from build123d import *

# Parameters (mm, degrees)
M10X1_0_TAPPED_HOLE1_D     = 9
M10X1_0_TAPPED_HOLE1_DEPTH = 28
M10X1_0_TAPPED_HOLE1_TIP   = 2.703872786
M4_TAPPED_HOLE1_D          = 3.3
M4_TAPPED_HOLE1_DEPTH      = 10.1
M4_TAPPED_HOLE1_TIP        = 0.991420021


with BuildPart() as part:
    # Sketch1 → Revolve1 (revolve)
    with BuildSketch(Plane.XY, mode=Mode.PRIVATE) as revolve1_sk:
        Polygon((0, 0), (-9, 0), (-9, 18), (-15, 36), (-15, 50), (-13.5, 50), (-13.5, 45), (0, 45), align=None)
    revolve(revolve1_sk.sketch.rotate(Axis((0, 0, 0), (0, -1, 0)), 270), axis=Axis((0, 0, 0), (0, -1, 0)))

    # M10x1.0 Tapped Hole1
    with Locations(Plane(origin=(0, 0, 0), x_dir=(-1, 0, 0), z_dir=(0, -1, 0))):
        with Locations((0, 0)):
            Hole(M10X1_0_TAPPED_HOLE1_D / 2, depth=M10X1_0_TAPPED_HOLE1_DEPTH)
            with Locations((0, 0, -(M10X1_0_TAPPED_HOLE1_DEPTH + M10X1_0_TAPPED_HOLE1_TIP / 2))):  # 118° drill point
                Cone(0, M10X1_0_TAPPED_HOLE1_D / 2, M10X1_0_TAPPED_HOLE1_TIP, mode=Mode.SUBTRACT)

    # M4 Tapped Hole1
    with Locations(Plane(origin=(0, 45, 0), x_dir=(1, 0, 0), z_dir=(0, 1, 0))):
        with Locations((0, 0)):
            Hole(M4_TAPPED_HOLE1_D / 2, depth=M4_TAPPED_HOLE1_DEPTH)
            with Locations((0, 0, -(M4_TAPPED_HOLE1_DEPTH + M4_TAPPED_HOLE1_TIP / 2))):  # 118° drill point
                Cone(0, M4_TAPPED_HOLE1_D / 2, M4_TAPPED_HOLE1_TIP, mode=Mode.SUBTRACT)


solid = part.part
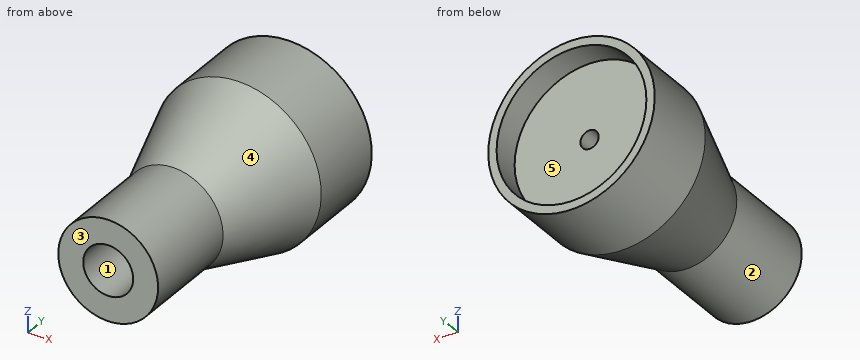
Source: CAD feature listing. Evaluate the final solid. Frame: model axes, mm. Face numbers are marked on the shaded views. A direction names the side the tool comes from. Coordinates: 2 decimals unless noted, no trailing zeros. Order: outer loops, then holes, each group sorted by start corner. A loop starts at its lowest first (then second) coordinate and runs counter-clockwise, first axis right, second up. Notation, with made-up numbers: M 40,55.25 L 79,55.25 A20 cw 79,74.25 Z; hole C -9.75,38.5 d3. An arc over 180 degrees is marked long. Write each question's results on one line, items separated by ' | '. Start each with the question number.
1. Pin query (flat end, axial travel): pin 1 (12 mm diameter, centred on y = 6.5, z = 11.5, fed in from +X); pin 2 (1 mm diameter, centred on x = 9.5, y = 23, fed in from +Z); pin 3 (8 mm diameter, centred on y = 11.5, z = 10.5, fed in from +X). Return the tip coordinate at first contact, or that it passes through.
2. Section B-B, the plane y = 37. Return the cut outline in (x, z).
3. Reachability of the marked faces 4 and 5 from +Z, -Z, +X, -X, +Y, -Y: full face, straight path, thin tool, end or side. Return the list, or none.
4. Draft query along X for the marked faces 1, 2 and 3. Return one class per face: +X half, -X half, draft (parallel to the pull), parting line (faces both ways), or undercut.
5. Section A-A, the plane y = 46. Return the cut outline in (x, z), then the cut area to 3 significant figures.
6. Material intervals for L1, parallel to Y at x = -1.5, z = 6.25; L2, parallel to X at y = 48.85, z = 0; L3, parallel to Z at x = 3.5, y = 47, sorted ascending.
Solution:
1) pin 1: x = 7.12 | pin 2: z = 5.78 | pin 3: x = 6.22
2) outline: C 0,0 d30; hole C 0,0 d3.3
3) face 4: -Y | face 5: +Y
4) face 1: undercut | face 2: parting line | face 3: draft
5) outline: C 0,0 d30; hole C 0,0 d27 | area: 134 mm²
6) L1: 0 to 45 | L2: -15 to -13.5, 13.5 to 15 | L3: -14.59 to -13.04, 13.04 to 14.59
